Check sheet for the drawn part. Datum: minimum x, y, z corner. Units: mm. Give positions to 0.01 mm unless a question says otherwise; leave off trailing zeros. Order: outer loops, then holes, each group sorted by start corner. A loop starts at its lowest first (then second) coordinate and runs counter-clockwise, first axis right, second up. Notation, with made-up numbers: (29, 67) -> (75, 67) arc R29 cw to (75, 95) -> close; hole circle Ø10 at (81, 2.25). An arc over 180 degrees is marked (long way). Answer in a Markdown table with one row per item. Add a question column.
(1) Go/stop test with a flat-tipped pin: pin 1 (4 mm diameter, centred on x = 47.5, z = 2, fed in from +Y). Record where the tip stops, or that it passes through.
(2) Release check for a two-part mould opening along X. For the marked faces 1, 2 and 3 record: released by +X, released by -X, zero draft, split by the parting line, or undercut.
(3) Cross-section at D-D (x = 61.5). Record the cut outline in (y, z).
(4) Cross-section at A-A (x = 40). Record the cut outline in (y, z), then the cut area to 3 significant figures.
(5) Cross-section at B-B (y = 62). Record the cut outline in (x, z), then the cut area to 3 significant figures.
(6) Cross-section at C-C (z = 1). Record the cut outline in (x, y), then the cut area to 3 significant figures.
(7) Thickness scan on L1, parallel to Y at x = 40, z = 5.5; L2, parallel to X at y = 59.5, z = 2.25; L3, parallel to X at y = 66, z = 3. Record the ranges inside material, lowest first. Write a range as [from, to].
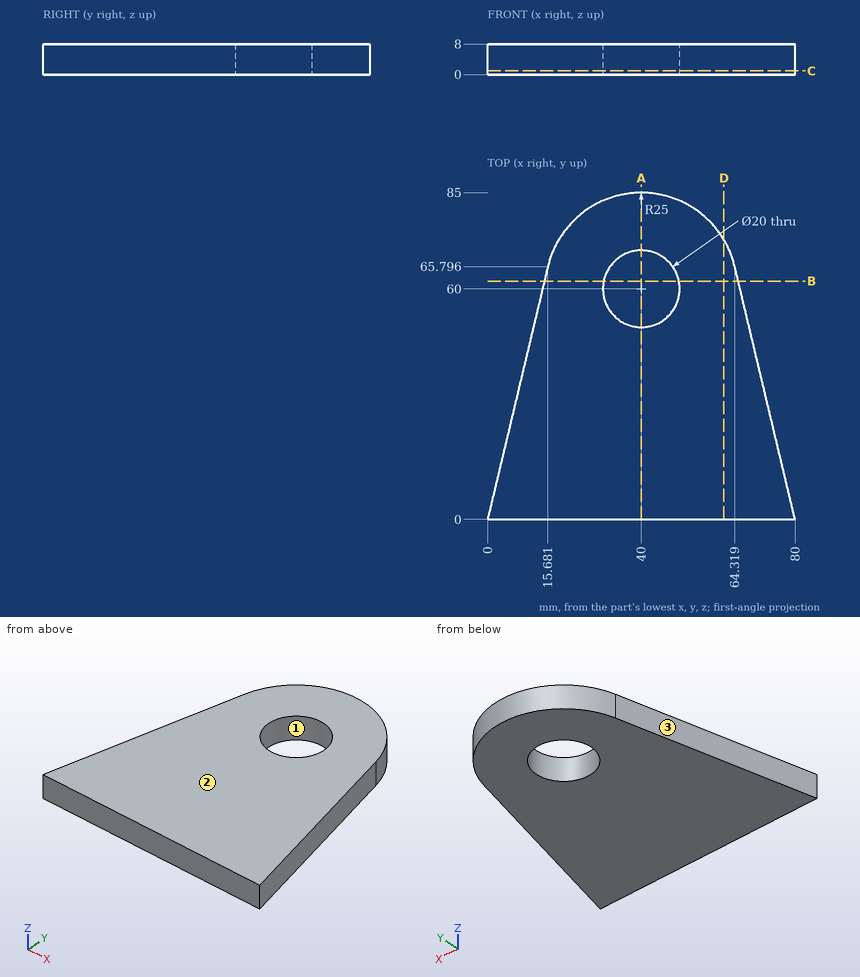
Answer below:
| question | item | result |
|---|---|---|
| 1 | pin 1 | stops at y = 84.39 |
| 2 | face 1 | undercut |
| 2 | face 2 | zero draft |
| 2 | face 3 | released by -X |
| 3 | outline | (0, 0) -> (72.76, 0) -> (72.76, 8) -> (0, 8) -> close |
| 4 | outline | (0, 0) -> (50, 0) -> (50, 8) -> (0, 8) -> close; (70, 0) -> (85, 0) -> (85, 8) -> (70, 8) -> close |
| 4 | area | 520 mm² |
| 5 | outline | (14.78, 0) -> (30.2, 0) -> (30.2, 8) -> (14.78, 8) -> close; (49.8, 0) -> (65.22, 0) -> (65.22, 8) -> (49.8, 8) -> close |
| 5 | area | 247 mm² |
| 6 | outline | (0, 0) -> (80, 0) -> (64.32, 65.8) arc R25 ccw to (15.68, 65.8) -> close; hole circle Ø20 at (40, 60) |
| 6 | area | 4,610 mm² |
| 7 | L1 | y = [0, 50], [70, 85] |
| 7 | L2 | x = [14.18, 30.01], [49.99, 65.82] |
| 7 | L3 | x = [15.73, 32], [48, 64.27] |
